Geometry: see drawing. Coordinates: mm, zero at the bounding-box minimum. Coordinates: 2 decimals unless noted, no trailing zeros. Write each loop counter-clockwise with the first axis right and the second up, starting at its lowest first coordinate (ties: lowest second). Pieces come first, ordered by that corner, then holes. Notation, with made-up numbers: M 15,57 L 51,57 A12 ccw 51,66 Z; hole C 87.25,27 d2. An arc over 180 degrees is marked long. One line per item, written item: value. Start each with the question number.
Item 1: Cut plane B-B, the plane z = 17.75. Output: boundary loops of the cut face in (x, y).
Item 2: Pin query (flat end, axial travel): P1, Ø13, axis at x = 218, y = 23, coming from the -Z side; P2, Ø2.5, axis at x = 239, z = 4.5, coming from the +Y side. Return the tip coordinate at first contact, or that it passes through.
Item 3: Ray query, L1, parallel to X at y = 24.5, z = 20; L2, parallel to Y at x = 422.5, z = 13.25; L3, parallel to Z at x = 445, y = 20. Return the intervals inside material, ascending. Write a range as from..to.
Item 4: Cut plane A-A, the plane x = 25. Output: boundary loops of the cut face in (y, z).
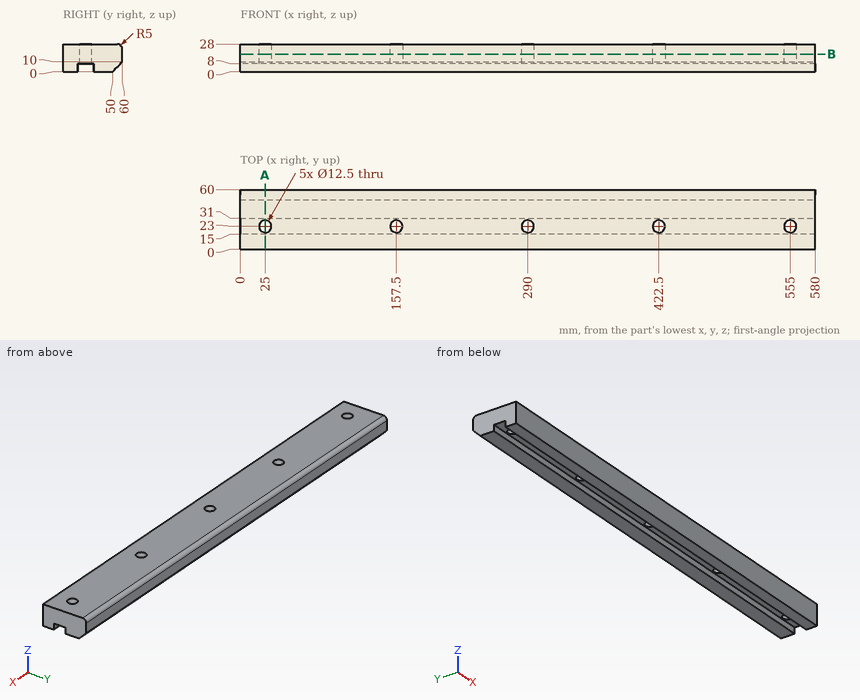
From the geometry:
1. outline: M 0,0 L 580,0 L 580,60 L 0,60 Z; hole C 25,23 d12.5; hole C 157.5,23 d12.5; hole C 290,23 d12.5; hole C 422.5,23 d12.5; hole C 555,23 d12.5
2. P1: stops at z = 8
2. P2: stops at y = 55.75
3. L1: x = 0..18.93, 31.07..151.43, 163.57..283.93, 296.07..416.43, 428.57..548.93, 561.07..580
3. L2: y = 0..16.75, 29.25..60
3. L3: z = 8..28
4. outline: M 0,0 L 15,0 L 15,8 L 16.75,8 L 16.75,28 L 0,28 Z; M 29.25,8 L 31,8 L 31,0 L 50,0 L 60,10 L 60,23 A5 ccw 55,28 L 29.25,28 Z
